from build123d import *

# Parameters (mm, degrees)
EXTRUDE_1_DEPTH        = 6
HOLE_WIZARD_M8_1_D     = 6.8
HOLE_WIZARD_M8_1_DEPTH = 15.75
HOLE_WIZARD_M8_1_TIP   = 2.042926105
HOLE_WIZARD_M4_1_D     = 3.3
PATTERN_LINEAR_1_COUNT = 3
PATTERN_LINEAR_1_PITCH = 160


with BuildPart() as part:
    # 草图1 → 凸台-拉伸1 (new, symmetric)
    with BuildSketch(Plane.XY):
        Polygon((180, -30), (195, -15), (195, 30), (-195, 30), (-195, -30), align=None)
        with BuildLine():
            Line((-177, 15), (-23, 15))
            ThreePointArc((-23, 15), (-20.878679656, 14.121320344), (-20, 12))
            Line((-20, 12), (-20, -15))
            ThreePointArc((-20, -15), (-20.878679656, -17.121320344), (-23, -18))
            Line((-23, -18), (-177, -18))
            ThreePointArc((-177, -18), (-179.121320344, -17.121320344), (-180, -15))
            Line((-180, -15), (-180, 12))
            ThreePointArc((-180, 12), (-179.121320344, 14.121320344), (-177, 15))
        make_face(mode=Mode.SUBTRACT)
        with BuildLine():
            Line((13, 15), (167, 15))
            ThreePointArc((167, 15), (169.121320344, 14.121320344), (170, 12))
            Line((170, 12), (170, -15))
            ThreePointArc((170, -15), (169.121320344, -17.121320344), (167, -18))
            Line((167, -18), (13, -18))
            ThreePointArc((13, -18), (10.878679656, -17.121320344), (10, -15))
            Line((10, -15), (10, 12))
            ThreePointArc((10, 12), (10.878679656, 14.121320344), (13, 15))
        make_face(mode=Mode.SUBTRACT)
    extrude(amount=EXTRUDE_1_DEPTH, both=True)

    # M8 螺纹孔1
    with Locations(Plane(origin=(-195, 20, 0), x_dir=(0, 0, -1), z_dir=(-1, 0, 0))):
        with Locations((0, 0), (0, 40)):
            Hole(HOLE_WIZARD_M8_1_D / 2, depth=HOLE_WIZARD_M8_1_DEPTH)
            with Locations((0, 0, -(HOLE_WIZARD_M8_1_DEPTH + HOLE_WIZARD_M8_1_TIP / 2))):  # 118° drill point
                Cone(0, HOLE_WIZARD_M8_1_D / 2, HOLE_WIZARD_M8_1_TIP, mode=Mode.SUBTRACT)

    # M4 螺纹孔1 (through all)
    with Locations(Plane.XY.offset(6)):
        with Locations((-15, -5), (5, -5)):
            Hole(HOLE_WIZARD_M4_1_D / 2)

    # 草图6 → M8 螺纹孔2 (revolve, cut)
    with BuildSketch(Plane(origin=(-145, 30, 0), x_dir=(0, 0, 1), z_dir=(1, 0, 0))):
        Polygon((0, 0), (0, 17.792926105), (3.4, 15.75), (3.4, 0), align=None)
    hole_wizard_m8_2 = revolve(axis=Axis((-145, 36.35, 0), (0, -1, 0)), mode=Mode.SUBTRACT)

    # 阵列(线性)1: M8 螺纹孔2 ×3
    with Locations(*[(i * PATTERN_LINEAR_1_PITCH, 0, 0) for i in range(1, PATTERN_LINEAR_1_COUNT)]):
        add(hole_wizard_m8_2, mode=Mode.SUBTRACT)


solid = part.part
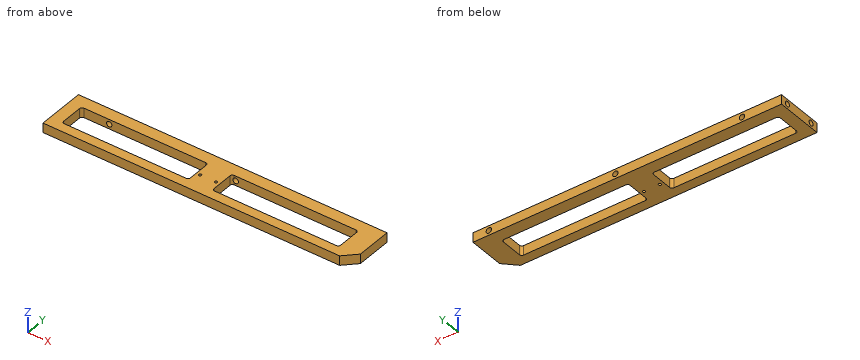
The model under review builds one solid part; all positions refer to its coordinate system, in mm. Give positions to 0.01 mm unless a question says otherwise; leave off trailing zeros. Loops run counter-clockwise (first coordinate to the right, second up) from the corner with the lowest first, then second, coordinate; pieces in that order, holes last. Notation, with made-up numbers: (-37, 49) -> (2, 49) arc R14 ccw to (2, 71) -> close; hole circle Ø5 at (76.25, -38.75). An arc over 180 degrees is marked (long way). Put each result on its own line as item: value. Start each with the question number.
1. Wall thickness on probe 1 along X at (y, z) = (7, -3.5); probe 2 along X at (y, z) = (-5.5, -2.25); probe 3 along Y at (x, z) = (110, -1): over which ranges is each line inside the solid? List them lowest first.
2. We need section A-A on x = -145. State the section outline as (y, z) points, then the cut area to 3 significant figures.
3. Clearance check with flat-ended pins moving along their axes: P1, Ø2, axis at y = 21.5, z = -1, coming from the -X side; P2, Ø4, axis at y = -20, z = 0, coming from the +X side; P3, Ø6, axis at x = 175, z = 0, coming from the +Y side. State where each tip first meets the part, or that it passes through.
4. We need section C-C on x = -76. State the section outline as (y, z) points.
5. We need section B-B on y = 2. State the section outline as (x, z) points.
Determined:
1. probe 1: -195 to -180, -20 to 10, 170 to 195
1. probe 2: -195 to -180, -20 to -16.57, -13.43 to 3.43, 6.57 to 10, 170 to 195
1. probe 3: -30 to -18, 15 to 30
2. outline: (-30, -6) -> (-18, -6) -> (-18, 6) -> (-30, 6) -> close; (15, -6) -> (30, -6) -> (30, -3.4) -> (15, -3.4) -> close; (15, 3.4) -> (30, 3.4) -> (30, 6) -> (15, 6) -> close
2. area: 222 mm^2
3. P1: x = -178.89
3. P2: x = 192
3. P3: y = 14.01
4. outline: (-30, -6) -> (-18, -6) -> (-18, 6) -> (-30, 6) -> close; (15, -6) -> (30, -6) -> (30, 6) -> (15, 6) -> close
5. outline: (-195, -6) -> (-180, -6) -> (-180, 6) -> (-195, 6) -> close; (-20, -6) -> (10, -6) -> (10, 6) -> (-20, 6) -> close; (170, -6) -> (195, -6) -> (195, 6) -> (170, 6) -> close
